from build123d import *

# Parameters (mm, degrees)
SKETCH1_W           = 365
SKETCH1_H           = 540
BOSS_EXTRUDE1_DEPTH = 8
M6_TAPPED_HOLE1_D   = 5
LPATTERN1_COUNT     = 6
LPATTERN1_PITCH     = 60


with BuildPart() as part:
    # Sketch1 → Boss-Extrude1 (new body)
    with BuildSketch(Plane.XY):
        with Locations((182.5, -270)):
            Rectangle(SKETCH1_W, SKETCH1_H)
        with BuildLine():
            Line((204.5, -39), (204.5, -179))
            ThreePointArc((204.5, -179), (182.5, -201), (160.5, -179))
            Line((160.5, -179), (160.5, -39))
            ThreePointArc((160.5, -39), (182.5, -17), (204.5, -39))
        make_face(mode=Mode.SUBTRACT)
    extrude(amount=BOSS_EXTRUDE1_DEPTH)

    # M6 Tapped Hole1 (through all)
    with Locations(Plane.XY.offset(8)):
        with Locations((79.5, -125), (285.5, -125)):
            m6_tapped_hole1 = Hole(M6_TAPPED_HOLE1_D / 2)

    # LPattern1: M6 Tapped Hole1 ×6
    with Locations(*[(0, -i * LPATTERN1_PITCH, 0) for i in range(1, LPATTERN1_COUNT)]):
        add(m6_tapped_hole1, mode=Mode.SUBTRACT)


solid = part.part
Can you work these out from the model? Positions are in its coordinate system, mm. A direction names the side the tool comes from. Give positions to 0.01 mm unless a question says otherwise; leave off trailing zeros. Order: outer loops, then holes, each group sorted by start corner. A loop starts at its lowest first (then second) coordinate and runs counter-clockwise, first axis right, second up. Notation, with made-up numbers: M 57.25,84 L 114.25,84 A15 cw 114.25,107 Z; hole C 81,61.25 d9. An arc over 180 degrees is marked long. Use one line per item in the form item = value.
Item 1: For faces 1 (the flat face through (180, -266, 0)), 2 (the cylindrical face through (182.984, -200.995, 3.944)), which set-ups out of +Z, -Z, +X, -X, +Y, -Y let a thin tool reach every point of the face, with its end or its side?
Values follow:
face_1 = -Z, +X, -X, +Y, -Y
face_2 = +Z, -Z
Item 2: Thinking about a two-plate mould opening in X: for faces 3 (the cylindrical face through (182.016, -17.005, 3.944)), 4 (the flat face through (180, -266, 8)), which applies, pulls with the +X half, pulls with the -X half, needs draft (parallel to the pull), parting line crosses it, or undercut?
Values follow:
face_3 = undercut
face_4 = needs draft
Item 3: If I drill on line 1 along X through (y, z) = (-425, 4.5); line 2 along X through (y, z) = (-184, 5.5); line 3 along X through (y, z) = (-80.5, 3.5), over which ranges is the centre line in solid material (lowest first)? Write a range as [from, to].
Values follow:
line_1 = [0, 77], [82, 283], [288, 365]
line_2 = [0, 77.21], [81.79, 161.08], [203.92, 283.21], [287.79, 365]
line_3 = [0, 160.5], [204.5, 365]
Item 4: If we section it at B-B, the plane z = 2: Count the separate pieces of the cut face and the enclosed holes in it, and give its area (3 significant figures).
Values follow:
separate_pieces = 1
enclosed_holes = 13
area = 189,000 mm^2
Item 5: If we section it at A-A, the plane x = 182.5: Write out the boundary of the cut face in (y, z), and give its area (3 significant figures).
Values follow:
outline = M -540,0 L -201,0 L -201,8 L -540,8 Z; M -17,0 L 0,0 L 0,8 L -17,8 Z
area = 2,850 mm^2
